Input: dimensioned drawing with shaded views. Units: mm. Origin: part minimum x, y, z. Coordinates: 2 decimals unless noted, no trailing zeros. Loops run counter-clockwise (first coordinate to the right, second up) from the corner with the lowest first, then second, coordinate; pieces in that order, holes last. Notation, with made-up numbers: M -31.5,29 L 24.5,29 A25 cw 24.5,48 Z; hole C 30,82.5 d5. An arc over 180 degrees is marked long. Write item = value, one per line. Start each with the question number.
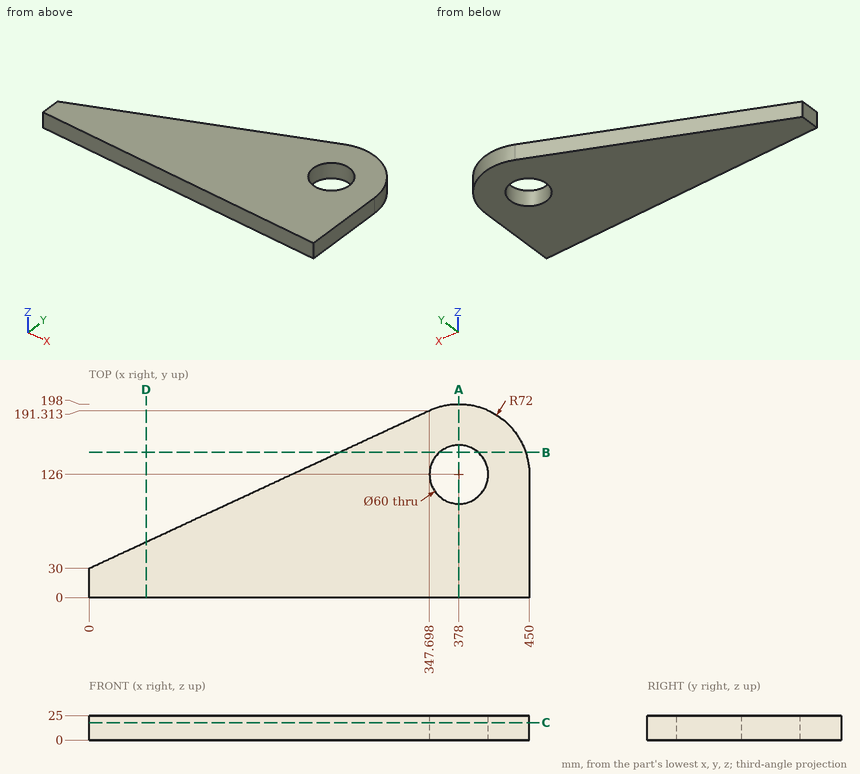
Item 1: Section query A-A (x = 378). Return the cut outline in (y, z), plus the area to 3 significant figures.
Item 2: Section query C-C (z = 18). Return the cut outline in (x, y).
Item 3: Section query D-D (x = 58.5). Return the cut outline in (y, z), plus the area to 3 significant figures.
Item 4: First-contact query: pin 1 (10 mm diameter, centred on y = 56, z = 10.5, fed in from -X) (1 decimal); pin 2 (1.5 mm diameter, centred on y = 138, z = 16, fed in from +X); pin 3 (3 mm diameter, centred on y = 51, z = 6, fed in from -X). Flat tips, straight axial feed; report the tip coordinate or a pass-through.
Item 5: Line query: line 1 (Y direction, x = 378, z = 5.75); line 2 (X direction, y = 115, z = 18.5); line 3 (X direction, y = 152.5, z = 13.25) (1 decimal). Output: solid intervals per line, ascending. Write a range as from..to.
Item 6: Section query B-B (y = 148.5). Return the cut outline in (x, z), plus the area to 3 significant figures.
Verdict:
q1.outline = M 0,0 L 96,0 L 96,25 L 0,25 Z; M 156,0 L 198,0 L 198,25 L 156,25 Z
q1.area = 3,450 mm2
q2.outline = M 0,0 L 450,0 L 450,126 A72 ccw 347.7,191.31 L 0,30 Z; hole C 378,126 d60
q3.outline = M 0,0 L 57.14,0 L 57.14,25 L 0,25 Z
q3.area = 1,430 mm2
q4.pin_1 = 45.3
q4.pin_2 = 449.12
q4.pin_3 = 42.03
q5.line_1 = 0..96, 156..198
q5.line_2 = 183.21..350.09, 405.91..450
q5.line_3 = 264..363.9, 392.1..444.9
q6.outline = M 255.42,0 L 358.16,0 L 358.16,25 L 255.42,25 Z; M 397.84,0 L 446.39,0 L 446.39,25 L 397.84,25 Z
q6.area = 3,780 mm2
